Geometry check sheet. Reference: drawing and pictorial views, mm from the part's lowest x, y, z. Round coordinates to 2 decimals unless told otherwise and drop trailing zeros. Write each loop counter-clockwise with the first axis right and the second up, starting at its lowest first coordinate (ties: lowest second). Pieces come first, ordered by that corner, then holes. Notation, with made-up numbers: M 58.25,18 L 112.25,18 A4 cw 112.25,25 Z; hole C 62.25,-8 d10. An arc over 180 degrees is marked long. Answer in a Markdown table with one row per item. Add a question column.
1. Material ranges on probe 1 along Z at (x, y) = (22.5, 7.5); probe 2 along X at (y, z) = (9, 22); probe 3 along Z at (x, y) = (25, 3.75), recorded low to high.
2. Sectioned sample at B-B on x = 22.5. Record the cut outline in (y, z).
3. Sectioned sample at C-C on y = 4.5. Record the cut outline in (x, z).
4. Sectioned sample at A-A on z = 22.5. Record the cut outline in (x, y), plus the area to 3 significant figures.
5. Go/stop test with flat-tipped pins: pin 1 Ø14.5 at (x, z) = (22.5, 22.5) entering from -Y; pin 2 Ø5 at (x, y) = (13.5, 8) entering from +Z; pin 3 Ø10 at (x, z) = (11.5, 40) entering from +Y; pin 4 Ø5 at (x, y) = (31.5, 4.5) entering from -Z. Record where each tip stops, or that it passes through.
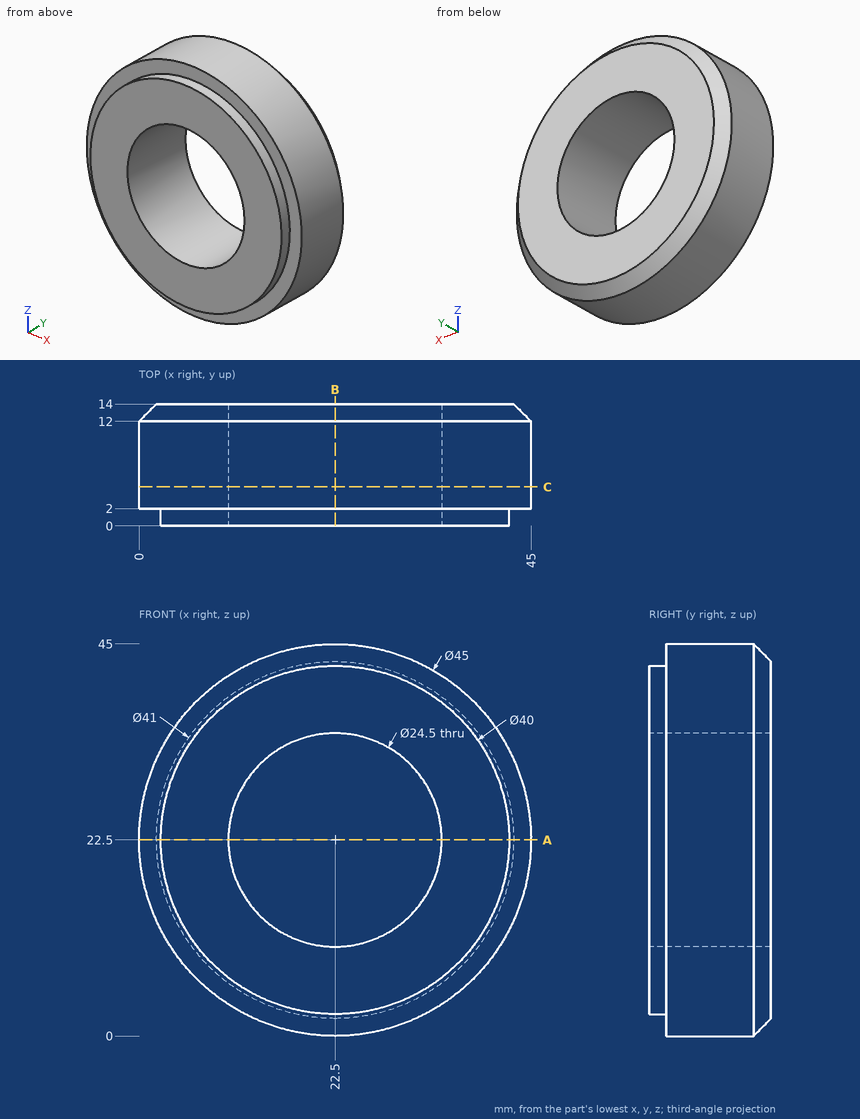
Geometry check:
| question | item | result |
|---|---|---|
| 1 | probe 1 | z = 0 to 10.25, 34.75 to 45 |
| 1 | probe 2 | x = 0.01 to 10.26, 34.74 to 44.99 |
| 1 | probe 3 | z = 0.14 to 10.51, 34.49 to 44.86 |
| 2 | outline | M 0,2.5 L 2,2.5 L 2,0 L 12,0 L 14,2 L 14,10.25 L 0,10.25 Z; M 0,34.75 L 14,34.75 L 14,43 L 12,45 L 2,45 L 2,42.5 L 0,42.5 Z |
| 3 | outline | C 22.5,22.5 d45; hole C 22.5,22.5 d24.5 |
| 4 | outline | M 0,2 L 2.5,2 L 2.5,0 L 10.25,0 L 10.25,14 L 2,14 L 0,12 Z; M 34.75,0 L 42.5,0 L 42.5,2 L 45,2 L 45,12 L 43,14 L 34.75,14 Z |
| 4 | area | 273 mm2 |
| 5 | pin 1 | passes through |
| 5 | pin 2 | stops at z = 44.04 |
| 5 | pin 3 | stops at y = 14 |
| 5 | pin 4 | stops at z = 0.96 |
